```python
from build123d import *

# Parameters (mm, degrees)
BOSS_EXTRUDE1_DEPTH     = 24
CUT_EXTRUDE1_DEPTH      = 47.914816423
CUT_EXTRUDE1_DEPTH_BACK = 47.914816423
SKETCH2_R               = 2
SKETCH3_W               = 40
SKETCH3_H               = 20
CUT_EXTRUDE2_DEPTH      = 48.707441768
SKETCH4_R               = 2
CUT_EXTRUDE3_DEPTH      = 47.914816423


with BuildPart() as part:
    # Sketch1 → Boss-Extrude1 (new body)
    with BuildSketch(Plane(origin=(0, 0, 0), x_dir=(1, 0, 0), z_dir=(0, 1, 0))):
        with BuildLine():
            Line((-5, 0), (-5, -40))
            Line((-5, -40), (5, -40))
            Line((5, -40), (5, 0))
            ThreePointArc((5, 0), (0, 5), (-5, 0))
        make_face()
    extrude(amount=BOSS_EXTRUDE1_DEPTH)

    # Sketch2 → Cut-Extrude1 (cut, two sides: drawn at the far end of the back side and taken through both)
    with BuildSketch(Plane(origin=(0, 24, 0), x_dir=(1, 0, 0), z_dir=(0, 1, 0)).offset(-CUT_EXTRUDE1_DEPTH_BACK)):
        with Locations(Location((0, 0, 0), (0, 0, 270))):
            Circle(SKETCH2_R)
    extrude(amount=CUT_EXTRUDE1_DEPTH + CUT_EXTRUDE1_DEPTH_BACK, mode=Mode.SUBTRACT)

    # Sketch3 → Cut-Extrude2 (cut, through all)
    with BuildSketch(Plane(origin=(5, 0, 0), x_dir=(0, 0, -1), z_dir=(1, 0, 0))):
        with Locations((-15, 12)):
            Rectangle(SKETCH3_W, SKETCH3_H)
    extrude(amount=-CUT_EXTRUDE2_DEPTH, mode=Mode.SUBTRACT)

    # Sketch4 → Cut-Extrude3 (cut, through all)
    with BuildSketch(Plane(origin=(0, 0, 35), x_dir=(-1, 0, 0), z_dir=(0, 0, -1))):
        with Locations((0, 12)):
            Circle(SKETCH4_R)
    extrude(amount=-CUT_EXTRUDE3_DEPTH, mode=Mode.SUBTRACT)


solid = part.part
```
For this review, take the finished solid that the model builds, in its own axes (mm). A direction names the side the tool comes from. Round coordinates to 2 decimals unless told otherwise and drop trailing zeros. Write each loop counter-clockwise with the first axis right and the second up, starting at its lowest first coordinate (ties: lowest second). Pieces come first, ordered by that corner, then holes. Notation, with made-up numbers: (38.5, 1) - (45.5, 1) arc R32 ccw to (45.5, 33) - close; hole circle Ø7 at (45, 24.5). An arc over 180 degrees is marked (long way). Use CSV: the item, a comma, the result in double quotes.
1) Clearance check with a flat-ended pin moving along its axis: pin 1 Ø5 at (x, y) = (1.5, 9) entering from -Z. State where the tip first meets the part, or that it passes through.
Conclusion:
pin 1,"stops at z = 35"
2) Add section A-A on x = 0. Write out the cut boundary in (y, z).
Conclusion:
outline,"(0, -5) - (2, -5) - (2, -2) - (0, -2) - close; (0, 2) - (2, 2) - (2, 35) - (10, 35) - (10, 40) - (0, 40) - close; (14, 35) - (22, 35) - (22, 2) - (24, 2) - (24, 40) - (14, 40) - close; (22, -5) - (24, -5) - (24, -2) - (22, -2) - close"
3) Add section B-B on z = 25. Write out the cut boundary in (x, y), and give its area (3 significant figures).
Conclusion:
outline,"(-5, 0) - (5, 0) - (5, 2) - (-5, 2) - close; (-5, 22) - (5, 22) - (5, 24) - (-5, 24) - close"
area,"40.0 mm^2"
4) For faces 4 (the flat face through (0, 22, 15)), 5 (the flat face through (-5, 11, 36)), list the 3-axis set-ups (+Z, -Z, +X, -X, +Y, -Y) from which the entire face can be reached by the end or side of a thin tool; tool diameter is ignored.
Conclusion:
face 4,"-Z, +X, -X"
face 5,"+Z, -Z, -X, +Y, -Y"
5) Add section C-C on y = 12. Write out the cut boundary in (x, z), and give its area (3 significant figures).
Conclusion:
outline,"(-5, 35) - (-2, 35) - (-2, 40) - (-5, 40) - close; (2, 35) - (5, 35) - (5, 40) - (2, 40) - close"
area,"30.0 mm^2"
6) Wall thickness on line 1 along Z through (x, y) = (0, 0.6); line 2 along Y through (x, z) = (-0.75, 14.5); line 3 along Z through (x, y) = (-4.25, 17.75): over which ranges is each line inside the solid? List them lowest first. Write a range as from..to.
Conclusion:
line 1,"z = -5..-2, 2..40"
line 2,"y = 0..2, 22..24"
line 3,"z = 35..40"
7) The part is to be moulded in two halves that separate along Y. For faces 1 (the flat face through (0, 2, 15)), 2 (the cylindrical face through (-2, 23, 0)), 3 (the flat face through (0, 24, 17)), say which applies: pulls with the +Y half, pulls with the -Y half, needs draft (parallel to the pull), parting line crosses it, or undercut.
Conclusion:
face 1,"undercut"
face 2,"needs draft"
face 3,"pulls with the +Y half"
8) Add section D-D on x = -3.25. Write out the cut boundary in (y, z), and give its area (3 significant figures).
Conclusion:
outline,"(0, -3.8) - (2, -3.8) - (2, 35) - (22, 35) - (22, -3.8) - (24, -3.8) - (24, 40) - (0, 40) - close"
area,"275 mm^2"
